The model under review builds one solid part; all positions refer to its coordinate system, in mm. A direction names the side the tool comes from. Give positions to 0.01 mm unless a question says otherwise; leave off trailing zeros. Write each loop counter-clockwise with the first axis right and the second up, starting at its lowest first coordinate (ties: lowest second). Pieces come first, ordered by that corner, then holes. Notation, with made-up numbers: M -33.5,89.5 L -3.5,89.5 A26 cw -3.5,128.5 Z; hole C -18.5,40.25 d9. An arc over 180 degrees is marked long. Write each question's results on one line, items separated by ' | '. Start each with the question number.
from build123d import *

# Parameters (mm, degrees)
BOSS_EXTRUDE1_DEPTH   = 20
CHAMFER1_SIZE         = 1
M6_TAPPED_HOLE1_D     = 5
M6_TAPPED_HOLE1_DEPTH = 9
M6_TAPPED_HOLE1_TIP   = 1.502151548
HOLE1_D               = 6.6
HOLE1_DEPTH           = 9
CHAMFER2_SIZE         = 1
FILLET1_R             = 5


with BuildPart() as part:
    # Sketch1 → Boss-Extrude1 (new body)
    with BuildSketch(Plane.XY):
        with BuildLine():
            Line((22.049935288, 34.795918367), (22.049935288, -25.204081633))
            Line((22.049935288, -25.204081633), (-47.950064712, -25.204081633))
            Line((-47.950064712, -25.204081633), (-47.950064712, -5.204081633))
            Line((-47.950064712, -5.204081633), (2.049935288, -5.204081633))
            Line((2.049935288, -5.204081633), (2.049935288, 34.795918367))
            Line((2.049935288, 34.795918367), (11.049935288, 34.795918367))
            Line((11.049935288, 34.795918367), (11.049935288, 25.71199815))
            ThreePointArc((11.049935288, 25.71199815), (12.049935288, 13.795918367), (13.049935288, 25.71199815))
            Line((13.049935288, 25.71199815), (13.049935288, 34.795918367))
            Line((13.049935288, 34.795918367), (22.049935288, 34.795918367))
        make_face()
        with BuildLine():
            Line((-40.450064712, -12.275048454), (-25.450064712, -12.275048454))
            ThreePointArc((-25.450064712, -12.275048454), (-22.521031533, -15.204081633), (-25.450064712, -18.133114812))
            Line((-25.450064712, -18.133114812), (-40.450064712, -18.133114812))
            ThreePointArc((-40.450064712, -18.133114812), (-43.379097891, -15.204081633), (-40.450064712, -12.275048454))
        make_face(mode=Mode.SUBTRACT)
        with BuildLine():
            Line((-5.450064712, -12.576085385), (9.549935288, -12.576085385))
            ThreePointArc((9.549935288, -12.576085385), (12.177931536, -15.204081633), (9.549935288, -17.832077881))
            Line((9.549935288, -17.832077881), (-5.450064712, -17.832077881))
            ThreePointArc((-5.450064712, -17.832077881), (-8.07806096, -15.204081633), (-5.450064712, -12.576085385))
        make_face(mode=Mode.SUBTRACT)
    extrude(amount=BOSS_EXTRUDE1_DEPTH)

    # Chamfer1
    chamfer1_edges = [part.edges().sort_by_distance(p)[0] for p in [
        (12.049935288, 13.795918367, 20),
        (12.049935288, 13.795918367, 0),
    ]]
    chamfer(chamfer1_edges, length=CHAMFER1_SIZE)

    # M6 Tapped Hole1
    with Locations(Plane.ZY.offset(-2.049935288)):
        with Locations((10, 30.295918367)):
            Hole(M6_TAPPED_HOLE1_D / 2, depth=M6_TAPPED_HOLE1_DEPTH)
            with Locations((0, 0, -(M6_TAPPED_HOLE1_DEPTH + M6_TAPPED_HOLE1_TIP / 2))):  # 118° drill point
                Cone(0, M6_TAPPED_HOLE1_D / 2, M6_TAPPED_HOLE1_TIP, mode=Mode.SUBTRACT)

    # Hole1
    with Locations(Plane(origin=(22.049935288, 0, 0), x_dir=(0, 0, -1), z_dir=(1, 0, 0))):
        with Locations((-10, 30.295918367)):
            Hole(HOLE1_D / 2, depth=HOLE1_DEPTH)

    # Chamfer2
    chamfer2_edges = [part.edges().sort_by_distance(p)[0] for p in [
        (22.049935288, 34.795918367, 10),
        (22.049935288, -25.204081633, 10),
        (-47.950064712, -25.204081633, 10),
        (-47.950064712, -5.204081633, 10),
        (2.049935288, 34.795918367, 10),
    ]]
    chamfer(chamfer2_edges, length=CHAMFER2_SIZE)

    # Fillet1
    fillet1_edges = [part.edges().sort_by_distance(p)[0] for p in [
        (2.049935288, -5.204081633, 10),
    ]]
    fillet(fillet1_edges, radius=FILLET1_R)


solid = part.part
(1) Machinability: for faces 4 (the flat face through (2, -17.832, 10)), 5 (the flat face through (2.05, 17, 10)), 6 (the flat face through (-5, -8, 0)), 7 (the flat face through (13.05, 27, 8)), 8 (the cylindrical face through (17.49, 32.53, 7.57)), which of the approach directions +Z, -Z, +X, -X, +Y, -Y give a long, thin tool a straight path to every point of the face, cutting with its end or side? Answer none if there is none.
(2) Add section C-C (y = -15). State the section outline as (x, z) points.
(3) Add section B-B (x = -31.5). State the section outline as (y, z) points.
(4) Wall thickness on L1, parallel to X at y = -15.5, z = 4.5; L2, parallel to X at y = -14, z = 8.25; L3, parallel to Y at x = 18.5, z = 10: over which ranges is each line inside the solid? List them lowest first.
(5) Draft analysis for pull direction Y (two halves, no side actions). For faces 1 (the flat face through (7, 34.796, 10)), 2 (the cylindrical face through (6.613, 30.406, 12.498)), 3 (the flat face through (-12, -25.204, 10)), state which applies: pulls with the +Y half, pulls with the -Y half, needs draft (parallel to the pull), parting line crosses it, or undercut.
(6) Add section A-A (z = 10). Give the number of separate pieces and of enclosed holes in the cut face, then the cut area to 3 significant figures.
(7) Add section D-D (y = 7). State the section outline as (x, z) points, then the cut area to 3 significant figures.
(8) Clearance check with flat-ended pins moving along their axes: P1, Ø7.5, axis at y = 29, z = 7, coming from the -X side; P2, Ø8, axis at x = -19, z = 9.5, coming from the +Y side. State where each tip first meets the part, or that it passes through.
Calculated:
1) face 4: +Z, -Z | face 5: +Z, -Z, -X, +Y | face 6: -Z, +X, -X, +Y, -Y | face 7: +Z, -Z, +Y | face 8: +X
2) outline: M -47.95,0 L -43.37,0 L -43.37,20 L -47.95,20 Z; M -22.53,0 L -8.07,0 L -8.07,20 L -22.53,20 Z; M 12.17,0 L 22.05,0 L 22.05,20 L 12.17,20 Z
3) outline: M -25.2,0 L -18.13,0 L -18.13,20 L -25.2,20 Z; M -12.28,0 L -5.2,0 L -5.2,20 L -12.28,20 Z
4) L1: x = -47.95 to -43.36, -22.54 to -8.06, 12.16 to 22.05 | L2: x = -47.95 to -43.12, -22.78 to -7.79, 11.89 to 22.05 | L3: y = -25.2 to 27, 33.6 to 34.8
5) face 1: pulls with the +Y half | face 2: undercut | face 3: pulls with the -Y half
6) separate pieces: 3 | enclosed holes: 2 | area: 1,750 mm²
7) outline: M 2.05,0 L 22.05,0 L 22.05,20 L 2.05,20 Z | area: 400 mm²
8) P1: stops at x = 2.05 | P2: stops at y = -5.2
